Input: part model. Units: mm. Frame: model coordinates. A direction names the side the tool comes from. Coordinates: 2 decimals unless noted, no trailing zeros. Order: outer loops, then holes, each group sorted by start corner. A loop starts at its lowest first (then second) coordinate and runs counter-clockwise, first axis right, second up. Notation, with made-up numbers: M -29,29.5 L -11,29.5 A29 ccw -11,59.5 Z; hole C 7.25,38 d1. An arc over 180 degrees is marked long. Answer in a Markdown table with one row per item.
from build123d import *

# Parameters (mm, degrees)
SKETCH1_W                      = 25
SKETCH1_H                      = 7
BOSS_EXTRUDE1_DEPTH            = 6
F_3_5_3_5_DIAMETER_HOLE2_D     = 3.5
F_3_5_3_5_DIAMETER_HOLE3_D     = 3.5
F_3_5_3_5_DIAMETER_HOLE3_DEPTH = 3
F_3_5_3_5_DIAMETER_HOLE3_TIP   = 1.051506083
CHAMFER1_SIZE                  = 0.5


with BuildPart() as part:
    # Sketch1 → Boss-Extrude1 (new body)
    with BuildSketch(Plane.XY):
        Rectangle(SKETCH1_W, SKETCH1_H)
    extrude(amount=BOSS_EXTRUDE1_DEPTH)

    # Ø3.5 (3.5) Diameter Hole2 (through all)
    with Locations(Plane.XY.offset(6)):
        with Locations((-10, 0.5), (10, 0.5)):
            Hole(F_3_5_3_5_DIAMETER_HOLE2_D / 2)

    # Ø3.5 (3.5) Diameter Hole3
    with Locations(Plane(origin=(0, 3.5, 0), x_dir=(1, 0, 0), z_dir=(0, 1, 0))):
        with Locations((5, -2.5), (-5, -2.5)):
            Hole(F_3_5_3_5_DIAMETER_HOLE3_D / 2, depth=F_3_5_3_5_DIAMETER_HOLE3_DEPTH)
            with Locations((0, 0, -(F_3_5_3_5_DIAMETER_HOLE3_DEPTH + F_3_5_3_5_DIAMETER_HOLE3_TIP / 2))):  # 118° drill point
                Cone(0, F_3_5_3_5_DIAMETER_HOLE3_D / 2, F_3_5_3_5_DIAMETER_HOLE3_TIP, mode=Mode.SUBTRACT)

    # Chamfer1
    chamfer1_edges = [part.edges().sort_by_distance(p)[0] for p in [
        (-12.5, 0, 6),
        (0, -3.5, 6),
        (12.5, 0, 6),
        (0, -3.5, 0),
        (-12.5, 0, 0),
        (0, 3.5, 0),
        (12.5, 0, 0),
        (0, 3.5, 6),
        (12.5, -3.5, 3),
        (-12.5, -3.5, 3),
        (-12.5, 3.5, 3),
        (12.5, 3.5, 3),
    ]]
    chamfer(chamfer1_edges, length=CHAMFER1_SIZE)


solid = part.part
1) Contact query for a flat-ended pin moving along its axis: pin 1 (2 mm diameter, centred on x = 10, y = 0.5, fed in from +Z). Output: stop coordinate, or through.
Resolved:
| item | result |
|---|---|
| pin 1 | passes through |
2) Cut plane D-D, the plane z = 3.3. State how many separate pieces and enclosed holes the cut face has, and give its area (3 significant figures).
Resolved:
| item | result |
|---|---|
| separate pieces | 1 |
| enclosed holes | 2 |
| area | 134 mm2 |
3) Cut plane C-C, the plane y = 2.5. Output: boundary loops of the cut face in (x, z), and give its area (3 significant figures).
Resolved:
| item | result |
|---|---|
| outline | M -12.5,0.5 L -12,0 L 12,0 L 12.5,0.5 L 12.5,5.5 L 12,6 L -12,6 L -12.5,5.5 Z; hole C -5,2.5 d3.5; hole C 5,2.5 d3.5 |
| area | 130 mm2 |
4) Cut plane A-A, the plane x = -10. Output: boundary loops of the cut face in (y, z).
Resolved:
| item | result |
|---|---|
| outline | M -3.5,0.5 L -3,0 L -1.25,0 L -1.25,6 L -3,6 L -3.5,5.5 Z; M 2.25,0 L 3,0 L 3.5,0.5 L 3.5,5.5 L 3,6 L 2.25,6 Z |
5) Material intervals for probe 1 along X at (y, z) = (-0.5, 1.8); probe 2 along X at (y, z) = (1.5, 4); probe 3 along X at (y, z) = (0, 2.2), sorted ascending.
Resolved:
| item | result |
|---|---|
| probe 1 | x = -12.5 to -11.44, -8.56 to 8.56, 11.44 to 12.5 |
| probe 2 | x = -12.5 to -11.44, -8.56 to -5.9, -4.1 to 4.1, 5.9 to 8.56, 11.44 to 12.5 |
| probe 3 | x = -12.5 to -11.68, -8.32 to -5.87, -4.13 to 4.13, 5.87 to 8.32, 11.68 to 12.5 |
6) Reachability of faces 1 (the face through (-3.25, 1.98, 2.42)), 2 (the face through (-11.669, 1.026, 2.958)) from +Z, -Z, +X, -X, +Y, -Y: full face, straight path, thin tool, end or side. Return the list, or none.
Resolved:
| item | result |
|---|---|
| face 1 | +Y |
| face 2 | +Z, -Z |
7) Cut plane B-B, the plane y = 0. Output: boundary loops of the cut face in (x, z).
Resolved:
| item | result |
|---|---|
| outline | M -12.5,0.5 L -12,0 L -11.68,0 L -11.68,6 L -12,6 L -12.5,5.5 Z; M -8.32,0 L 8.32,0 L 8.32,6 L -8.32,6 Z; M 11.68,0 L 12,0 L 12.5,0.5 L 12.5,5.5 L 12,6 L 11.68,6 Z; hole C -5,2.5 d1.84; hole C 5,2.5 d1.84 |
8) Mould query, pull axis Z, two halves, no side actions, for faces 3 (the face through (6.75, 1.98, 2.42)), 4 (the face through (0, 0, 0)), 5 (the face through (0, 3.5, 3)). Classes: +Z half, -Z half, draft (parallel to the pull), parting line (faces both ways), or undercut.
Resolved:
| item | result |
|---|---|
| face 3 | undercut |
| face 4 | -Z half |
| face 5 | draft |
